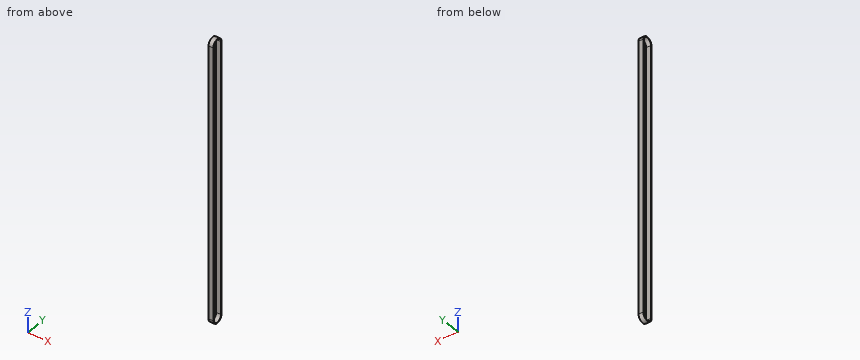
from build123d import *

# Parameters (mm, degrees)
EXTRUDE_1_DEPTH = 15


with BuildPart() as part:
    # 草图2 → 拉伸-薄壁1 (new, symmetric)
    with BuildSketch(Plane(origin=(0, 0, 0), x_dir=(0, 0, -1), z_dir=(1, 0, 0))):
        with BuildLine():
            Line((-1740, -35.35), (0, -35.35))
            ThreePointArc((0, -35.35), (35.35, 0), (0, 35.35))
            Line((0, 35.35), (-1740, 35.35))
            ThreePointArc((-1740, 35.35), (-1775.35, 0), (-1740, -35.35))
        make_face()
        with BuildLine():
            Line((-1740, -30.85), (0, -30.85))
            ThreePointArc((0, -30.85), (30.85, 0), (0, 30.85))
            Line((0, 30.85), (-1740, 30.85))
            ThreePointArc((-1740, 30.85), (-1770.85, 0), (-1740, -30.85))
        make_face(mode=Mode.SUBTRACT)
    extrude(amount=EXTRUDE_1_DEPTH, both=True)


solid = part.part
Source: CAD feature listing. Evaluate the final solid. Frame: model axes, mm. Round coordinates to 2 decimals unless told otherwise and drop trailing zeros. Write each loop counter-clockwise with the first axis right and the second up, starting at its lowest first coordinate (ties: lowest second). Pieces come first, ordered by that corner, then holes. Notation, with made-up numbers: (-4.5, -26) - (30.5, -26) arc R16 cw to (30.5, 1) - close; hole circle Ø8 at (84.25, 11). An arc over 180 degrees is marked (long way). Use CSV: the item, a comma, the result in double quotes. Start each with the question number.
(1) Cut plane B-B, the plane y = -16. Return loops of the section in (x, z), and give its area (3 significant figures).
(2) Material intervals for probe 1 along Y at (x, z) = (4.25, 1576); probe 2 along Z at (x, y) = (2.5, 3), sorted ascending. Write a range as [from, to].
(3) Cut plane A-A, the plane z = 496. Return loops of the section in (x, y), and give its area (3 significant figures).
(4) First-contact query: pin 1 Ø4 at (x, y) = (8, 11) entering from +Z; pin 2 Ø8 at (x, y) = (4.5, 20) entering from -Z; pin 3 Ø1 at (x, y) = (-9, -27.5) entering from +Z; pin 4 Ø6 at (y, z) = (-25, 942.5) entering from +X. Flat tips, straight axial feed; report the tip coordinate or a pass-through.
(5) Cut plane C-C, the plane x = -7.25. Return loops of the section in (y, z), and give its area (3 significant figures).
Geometry says:
1,outline,"(-15, -31.52) - (15, -31.52) - (15, -26.38) - (-15, -26.38) - close; (-15, 1766.38) - (15, 1766.38) - (15, 1771.52) - (-15, 1771.52) - close"
1,area,"309 mm²"
2,probe 1,"[-35.35, -30.85], [30.85, 35.35]"
2,probe 2,"[-35.22, -30.7], [1770.7, 1775.22]"
3,outline,"(-15, -35.35) - (15, -35.35) - (15, -30.85) - (-15, -30.85) - close; (-15, 30.85) - (15, 30.85) - (15, 35.35) - (-15, 35.35) - close"
3,area,"270 mm²"
4,pin 1,"z = 1774.19"
4,pin 2,"z = -31.52"
4,pin 3,"z = 1762.82"
4,pin 4,"through"
5,outline,"(-35.35, 0) arc R35.35 ccw to (35.35, 0) - (35.35, 1740) arc R35.35 ccw to (-35.35, 1740) - close; hole (-30.85, 0) arc R30.85 ccw to (30.85, 0) - (30.85, 1740) arc R30.85 ccw to (-30.85, 1740) - close"
5,area,"16,600 mm²"
